Could you check a few things on this drawing? It's one solid part, dimensions in mm from its lowest x, y, z. A direction names the side the tool comes from. Coordinates: 2 decimals unless noted, no trailing zeros. Order: outer loops, then holes, each group sorted by start corner. A loop starts at its lowest first (then second) coordinate and runs counter-clockwise, first axis right, second up.
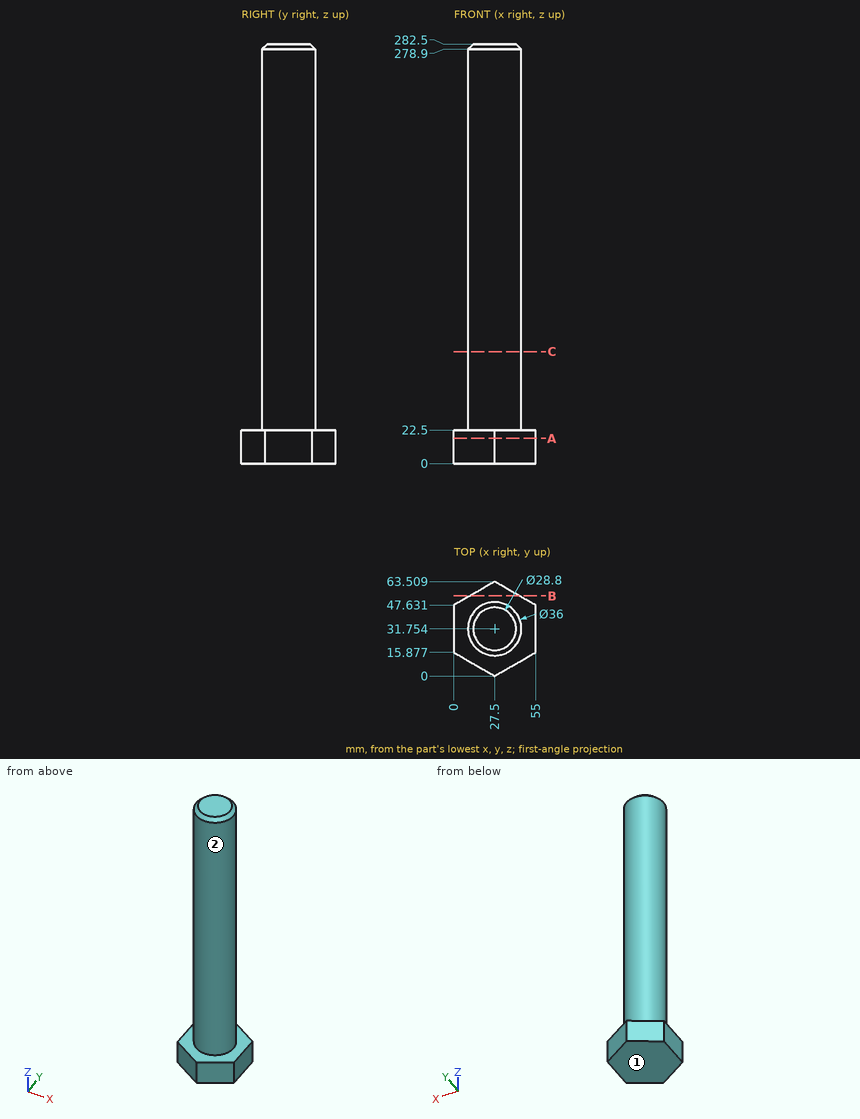
1. On a 3-axis mill with a long thin cutter (end or side, diameter ignored), from which of +Z, -Z, +X, -X, +Y, -Y can I reach the whole of each face in a straight line? I mean the marked faces 1 and 2. Say none if no direction works.
Completed:
face 1: -Z, +X, -X, +Y, -Y
face 2: +Z
2. Please list where these lines run through material, in increasing order: probe 1 along Z at (x, y) = (14, 17); probe 2 along X at (y, z) = (32.5, 156.5) (1 decimal); probe 3 along Y at (x, z) = (28, 34.5).
Completed:
probe 1: z = 0 to 22.5
probe 2: x = 9.5 to 45.5
probe 3: y = 13.76 to 49.75
3. Imagine slicing it at B-B on y = 54. Please give me the cut outline in (x, z), then the cut area to 3 significant figures.
Completed:
outline: (11.03, 0) - (43.97, 0) - (43.97, 22.5) - (11.03, 22.5) - close
area: 741 mm2
4. I'm going to push flat-ended pins straight in: pin 1 (3 mm diameter, centred on x = 39.5, y = 41.5, fed in from -Z); pin 2 (1.5 mm diameter, centred on x = 43.5, z = 204, fed in from -Y). Where does each tip first touch, or does it pass through?
Completed:
pin 1: stops at z = 0
pin 2: stops at y = 22.19
5. Imagine slicing it at A-A on z = 17. Please give me the cut outline in (x, y).
Completed:
outline: (0, 15.88) - (27.5, 0) - (55, 15.88) - (55, 47.63) - (27.5, 63.51) - (0, 47.63) - close
6. Imagine slicing it at C-C on z = 75.5. Please give me the cut outline in (x, y) (1 decimal), then the cut area to 3 significant figures.
Completed:
outline: circle Ø36 at (27.5, 31.8)
area: 1,020 mm2
